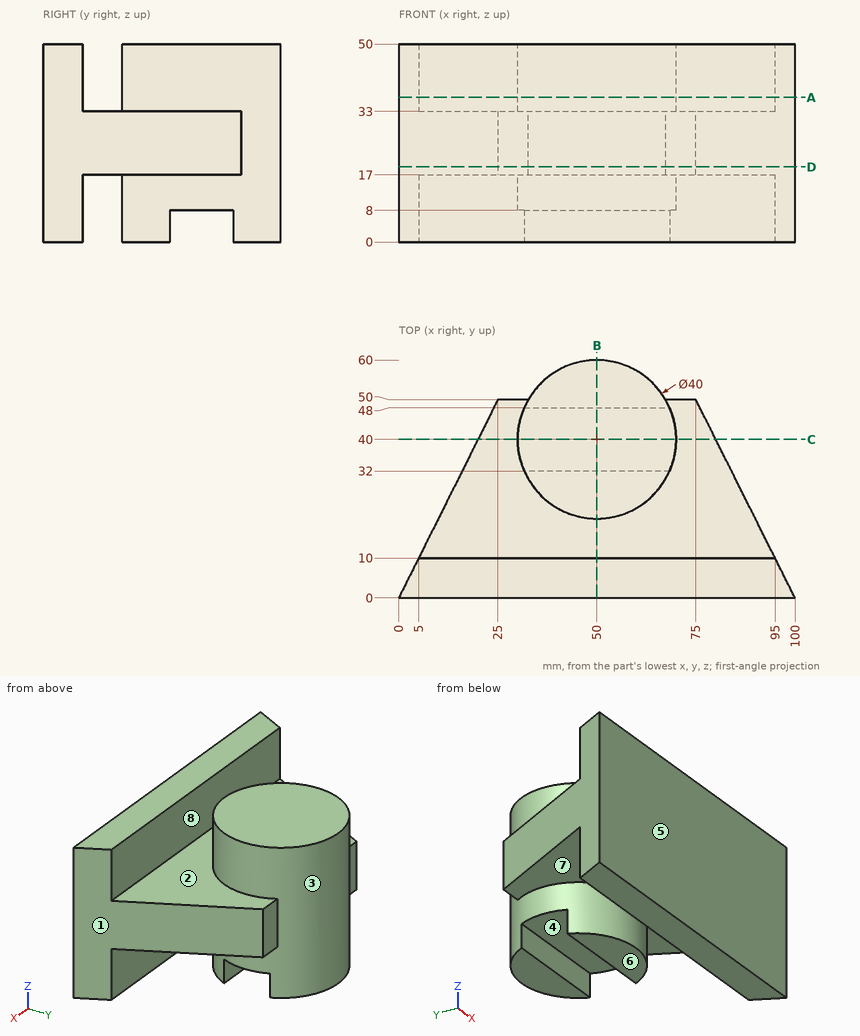
Job drawing, mm, ordinate dimensions from the low corner. One solid piece. A direction names the side the tool comes from. Coordinates: 2 decimals unless noted, no trailing zeros. Order: outer loops, then holes, each group sorted by start corner. A loop starts at its lowest first (then second) coordinate and runs counter-clockwise, first axis right, second up. Notation, with made-up numbers: M -34.5,43.25 L 14.5,43.25 A7 ccw 14.5,48.25 Z; hole C 77,21.5 d2. An arc over 180 degrees is marked long. Return JSON: item names as keys, results as strings.
1. Tool access for the marked faces 1, 2, 3 and 4: list every direction of +Z, -Z, +X, -X, +Y, -Y with a clear straight run to the whole face (end or side of a thin tool).
Ans:
{"face 1": "+Z, -Z, +X, +Y", "face 2": "+Z", "face 3": "none", "face 4": "-Z, +X, -X"}
2. Flat gauge pins, fed straight in: pin 1 (1 mm diameter, centred on y = 12, z = 10.5, fed in from +X); pin 2 (4 mm diameter, centred on x = 23, y = 35.5, fed in from +Z); pin 3 (17.5 mm diameter, centred on x = 53, y = 37.5, fed in from -Z); pin 4 (6 mm diameter, centred on x = 73, z = 28, fed in from +Y). Where does each tip first touch, or does it go through?
Ans:
{"pin 1": "through", "pin 2": "z = 33", "pin 3": "z = 0", "pin 4": "y = 50"}
3. Saw through at B-B (x = 50). Give the cut face in (y, z).
Ans:
{"outline": "M 0,0 L 10,0 L 10,17 L 20,17 L 20,0 L 32,0 L 32,8 L 48,8 L 48,0 L 60,0 L 60,50 L 20,50 L 20,33 L 10,33 L 10,50 L 0,50 Z"}
4. Saw through at D-D (z = 19). Give the cut face in (x, y), and give its area (3 significant figures).
Ans:
{"outline": "M 0,0 L 100,0 L 75,50 L 67.32,50 A20 ccw 32.68,50 L 25,50 Z", "area": "4,000 mm^2"}
5. Saw through at A-A (z = 36.5). Give the cut face in (x, y), and give its area (3 significant figures).
Ans:
{"outline": "M 0,0 L 100,0 L 95,10 L 5,10 Z; C 50,40 d40", "area": "2,210 mm^2"}
6. Saw through at C-C (y = 40). Give the cut face in (x, z).
Ans:
{"outline": "M 20,17 L 30,17 L 30,8 L 70,8 L 70,17 L 80,17 L 80,33 L 70,33 L 70,50 L 30,50 L 30,33 L 20,33 Z"}
7. Pull direction Y, two halves, no side cores. Call the marked faces 5, 6, 7 and 8: +Y half, -Y half, draft (parallel to the pull), parting line (faces both ways), or undercut.
Ans:
{"face 5": "-Y half", "face 6": "draft", "face 7": "undercut", "face 8": "undercut"}
8. Drill centre lines: probe 1 along Y at (x, z) = (50, 7.5); probe 2 along Y at (x, z) = (37.5, 2); probe 3 along Y at (x, z) = (30.5, 24.5). Where is each one in solid material? Low to high.
Ans:
{"probe 1": "0 to 10, 20 to 32, 48 to 60", "probe 2": "0 to 10, 24.39 to 32, 48 to 55.61", "probe 3": "0 to 50"}
